The listing builds one solid part. Answer for the finished solid, in the listing's coordinates (mm). A direction names the side the tool comes from. Round coordinates to 2 decimals unless told otherwise and drop trailing zeros. Write each loop counter-clockwise with the first axis right and the second up, starting at its lowest first coordinate (ties: lowest second). Pieces come first, ordered by that corner, then holes. Notation, with made-up numbers: M -19,-22.5 L 3,-22.5 A27 ccw 3,-3.5 Z; hole C 51.5,-27.5 d10. An arc over 180 degrees is marked long. One line per item, written item: value. Start each with the question number.
(1) Section D-D (y = 24.5) is taken. Determine the outline of the cut face in (x, z).
(2) Section C-C (x = 16) is taken. Determine the outline of the cut face in (y, z), plus the area to 3 significant figures.
(3) For a pull along X with two mould halves and no side action, classify faces 4 (the flat face through (42, 32, 0)), 5 (the flat face through (1, 0, 1)), 6 (the flat face through (9.5, 72, 0)) as released by +X, released by -X, zero draft, split by the parting line, or undercut.
(4) Section B-B (z = 7.5) is taken. Determine the outline of the cut face in (x, y).
(5) Consider probe 1 along Z at (x, y) = (-32.5, 82); probe 2 along Y at (x, z) = (-1.5, -0.5); probe 3 along Y at (x, z) = (-11, 27.5). Determine where each line is inside the solid, lowest interval first.
(6) Section A-A (y = 77.5) is taken. Determine the outline of the cut face in (x, z), plus the area to 3 significant figures.
(7) Given P1, Ø5, axis at x = 12.5, z = -34.5, coming from the +Y side; P2, Ø1.5, axis at x = -13, z = 26.5, coming from the -Y side; P3, Ø6, axis at x = 10, y = 19.5, coming from the -Z side; P4, Ø5, axis at x = -17.5, z = 55.5, coming from the +Y side, each flat-ended and moving along its own axis, determine where each tip first touches the part or whether it passes through.
(8) For faces 1 (the flat face through (1, 32, -30)), 2 (the flat face through (-9.5, 73, 0)), 3 (the flat face through (-5, 22, 44)), determine the directions among +Z, -Z, +X, -X, +Y, -Y from which every point of the face is accessible in a straight line to the end or side of a thin tool.
```python
from build123d import *

# Parameters (mm, degrees)
BRACKET_BODY_DEPTH            = 42
UPRIGHT_PROFILE_CUT_DEPTH     = 40
GUIDE_SLOT_DEPTH              = 40
ANGLED_CORNER_CUT_39DEG_DEPTH = 40


with BuildPart() as part:
    # Bracket Side Profile Sketch → Bracket Body (new, symmetric)
    with BuildSketch(Plane(origin=(0, 0, 0), x_dir=(0, 0, -1), z_dir=(1, 0, 0))):
        Polygon((-60, 0), (60, 0), (60, 12), (44, 12), (44, 32), (16, 32), (16, 124), (-16, 124), (-16, 32), (-44, 32), (-44, 12), (-60, 12), align=None)
    extrude(amount=BRACKET_BODY_DEPTH, both=True)

    # Upright Profile Cut Sketch → Upright Profile Cut (cut)
    with BuildSketch(Plane(origin=(0, 0, -16), x_dir=(-1, 0, 0), z_dir=(0, 0, -1))):
        with BuildLine():
            Line((-42, 124), (-42, 82))
            ThreePointArc((-42, 82), (-29.69848481, 111.69848481), (0, 124))
            Line((0, 124), (-42, 124))
        make_face()
        with BuildLine():
            Line((42, 124), (0, 124))
            ThreePointArc((0, 124), (29.69848481, 111.69848481), (42, 82))
            Line((42, 82), (42, 124))
        make_face()
    extrude(amount=-UPRIGHT_PROFILE_CUT_DEPTH, mode=Mode.SUBTRACT)

    # Guide Slot Sketch → Guide Slot (cut)
    with BuildSketch(Plane(origin=(0, 0, -16), x_dir=(-1, 0, 0), z_dir=(0, 0, -1))):
        with BuildLine():
            Line((9.5, 82), (9.5, 63))
            ThreePointArc((9.5, 63), (0, 53.5), (-9.5, 63))
            Line((-9.5, 63), (-9.5, 82))
            ThreePointArc((-9.5, 82), (0, 91.5), (9.5, 82))
        make_face()
    extrude(amount=-GUIDE_SLOT_DEPTH, mode=Mode.SUBTRACT)

    # Angled Corner Cut Sketch 39deg → Angled Corner Cut 39deg (cut)
    with BuildSketch(Plane(origin=(0, 32, 0), x_dir=(1, 0, 0), z_dir=(0, 1, 0))):
        Polygon((42, 30), (17.706479004, 60), (42, 60), align=None)
        Polygon((42, -60), (42, -30), (17.706479004, -60), align=None)
    extrude(amount=-ANGLED_CORNER_CUT_39DEG_DEPTH, mode=Mode.SUBTRACT)


solid = part.part
```
Recorded:
1. outline: M -42,-44 L 30.66,-44 L 42,-30 L 42,30 L 30.66,44 L -42,44 Z
2. outline: M 0,-60 L 12,-60 L 12,-44 L 32,-44 L 32,-16 L 120.83,-16 L 120.83,16 L 32,16 L 32,44 L 12,44 L 12,60 L 0,60 Z
2. area: 6,040 mm2
3. face 4: released by +X
3. face 5: zero draft
3. face 6: undercut
4. outline: M -42,0 L 42,0 L 42,82 A42 ccw -42,82 Z; hole M -9.5,63 A9.5 ccw 9.5,63 L 9.5,82 A9.5 ccw -9.5,82 Z
5. probe 1: z = -16 to 16
5. probe 2: y = 0 to 53.62, 91.38 to 123.97
5. probe 3: y = 0 to 32
6. outline: M -42,-16 L -9.5,-16 L -9.5,16 L -42,16 Z; M 9.5,-16 L 42,-16 L 42,16 L 9.5,16 Z
6. area: 2,080 mm2
7. P1: stops at y = 32
7. P2: stops at y = 0
7. P3: stops at z = -44
7. P4: stops at y = 12
8. face 1: -Z, +X, -X, +Y
8. face 2: +Z, -Z
8. face 3: +Z, +X, -X, +Y
